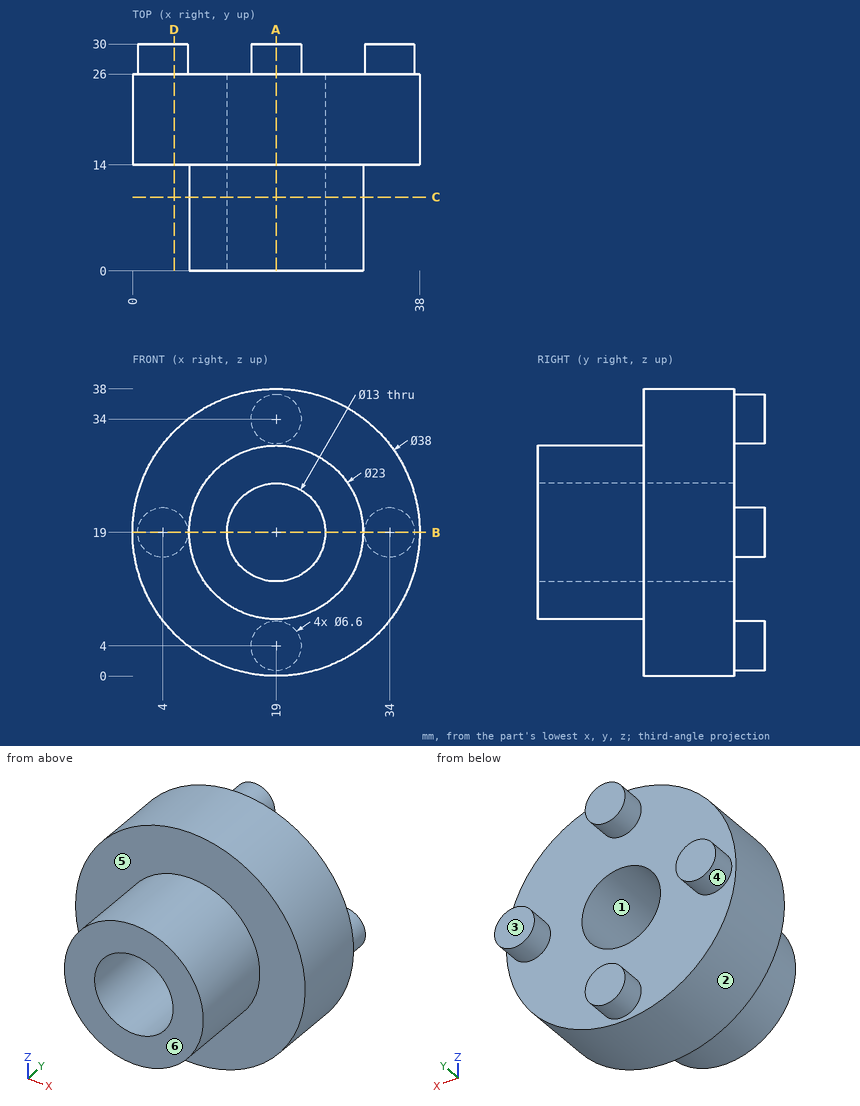
Job drawing, mm, ordinate dimensions from the low corner. One solid piece. A direction names the side the tool comes from. Coordinates: 2 decimals unless noted, no trailing zeros. Order: outer loops, then holes, each group sorted by start corner. A loop starts at its lowest first (then second) coordinate and runs counter-clockwise, first axis right, second up. Notation, with made-up numbers: (8.5, 62.25) - (27.5, 62.25) arc R22 ccw to (27.5, 74.25) - close; hole circle Ø3 at (-18.5, 63). An arc over 180 degrees is marked (long way). Return JSON: item names as keys, results as strings. Group by question number.
1) Saw through at B-B, the plane z = 19. Write the cut outline in (x, y), plus the area to 3 significant figures.
2) Saw through at D-D, the plane x = 5.5. Write the cut outline in (y, z).
3) Mould opens along Z. For the marked faces 1, 2 and 3 say: released by +Z, released by -Z, zero draft, split by the parting line, or undercut.
4) Saw through at C-C, the plane y = 9.75. Write the cut outline in (x, z).
5) Tool access for the marked faces 4, 5 and 6: list every direction of +Z, -Z, +X, -X, +Y, -Y with a clear straight run to the whole face (end or side of a thin tool).
6) Saw through at A-A, the plane x = 19. Write the cut outline in (y, z).
7) Probe line 1 (X direction, y = 17.5, z = 19); line 2 (Y direction, x = 3, z = 11.5); line 3 (Y direction, x = 35, z = 16). List the from-to ranges inside material, lowest first. Write a range as from..to.
8) Flat gauge pins, fed straight in: P1, Ø2, axis at x = 12.5, z = 26, coming from the +Y side; P2, Ø10, axis at x = 23, y = 25.5, coming from the -Z side; P3, Ø3, axis at y = 24.5, z = 21.5, coming from the +X side; P4, Ø10, axis at x = 9, y = 21, coming from the -Z side. Where does each tip first touch, or does it go through?
Values found:
{
 "1": {"outline": "(0, 14) - (7.5, 14) - (7.5, 0) - (12.5, 0) - (12.5, 26) - (7.3, 26) - (7.3, 30) - (0.7, 30) - (0.7, 26) - (0, 26) - close; (25.5, 0) - (30.5, 0) - (30.5, 14) - (38, 14) - (38, 26) - (37.3, 26) - (37.3, 30) - (30.7, 30) - (30.7, 26) - (25.5, 26) - close", "area": "493 mm²"},
 "2": {"outline": "(14, 5.63) - (26, 5.63) - (26, 16.06) - (30, 16.06) - (30, 21.94) - (26, 21.94) - (26, 32.37) - (14, 32.37) - close"},
 "3": {"face 1": "undercut", "face 2": "split by the parting line", "face 3": "zero draft"},
 "4": {"outline": "circle Ø23 at (19, 19); hole circle Ø13 at (19, 19)"},
 "5": {"face 4": "+Y", "face 5": "-Y", "face 6": "+Z, -Z, +X, -X, -Y"},
 "6": {"outline": "(0, 7.5) - (14, 7.5) - (14, 0) - (26, 0) - (26, 0.7) - (30, 0.7) - (30, 7.3) - (26, 7.3) - (26, 12.5) - (0, 12.5) - close; (0, 25.5) - (26, 25.5) - (26, 30.7) - (30, 30.7) - (30, 37.3) - (26, 37.3) - (26, 38) - (14, 38) - (14, 30.5) - (0, 30.5) - close"},
 "7": {"line 1": "x = 0..12.5, 25.5..38", "line 2": "y = 14..26", "line 3": "y = 14..30"},
 "8": {"P1": "stops at y = 26", "P2": "stops at z = 0", "P3": "stops at x = 37.97", "P4": "stops at z = 0.67"}
}
